Geometry check sheet. Reference: the model listing, model coordinates, mm. Coordinates: 2 decimals unless noted, no trailing zeros. Loops run counter-clockwise (first coordinate to the right, second up) from the corner with the lowest first, then second, coordinate; pieces in that order, holes last. Notation, with made-up numbers: M 18.25,53.25 L 45.25,53.25 A19 ccw 45.25,70.25 Z; hole C 48,20.25 d4. An arc over 180 degrees is marked long. Use CSV: the item, a comma, the result in double quotes.
```python
from build123d import *

# Parameters (mm, degrees)
SKETCH1_W              = 900
SKETCH1_H              = 110
BOSS_EXTRUDE1_DEPTH    = 30
CHAMFER1_SIZE          = 10
CHAMFER2_SIZE          = 15
CHAMFER2_SIZE2         = 10
M16_TAPPED_HOLE1_D     = 14
M16_TAPPED_HOLE1_DEPTH = 45
M16_TAPPED_HOLE1_TIP   = 4.206024333


with BuildPart() as part:
    # Sketch1 → Boss-Extrude1 (new body)
    with BuildSketch(Plane.XY):
        with Locations((450, 55)):
            Rectangle(SKETCH1_W, SKETCH1_H)
    extrude(amount=BOSS_EXTRUDE1_DEPTH)

    # Chamfer1
    chamfer1_edges = [part.edges().sort_by_distance(p)[0] for p in [
        (450, 110, 30),
        (450, 0, 30),
    ]]
    chamfer(chamfer1_edges, length=CHAMFER1_SIZE)

    # Chamfer2
    chamfer2_edges = [part.edges().sort_by_distance(p)[0] for p in [
        (0, 55, 30),
    ]]
    chamfer2_side = [part.faces().sort_by_distance(p)[0] for p in [
        (0, 55, 14.635416667),
    ]]
    chamfer(chamfer2_edges, length=CHAMFER2_SIZE, length2=CHAMFER2_SIZE2, reference=chamfer2_side[0])

    # M16 Tapped Hole1
    with Locations(Plane(origin=(900, 55, 15), x_dir=(0, 0, 1), z_dir=(1, 0, 0))):
        with Locations((0, 0)):
            Hole(M16_TAPPED_HOLE1_D / 2, depth=M16_TAPPED_HOLE1_DEPTH)
            with Locations((0, 0, -(M16_TAPPED_HOLE1_DEPTH + M16_TAPPED_HOLE1_TIP / 2))):  # 118° drill point
                Cone(0, M16_TAPPED_HOLE1_D / 2, M16_TAPPED_HOLE1_TIP, mode=Mode.SUBTRACT)


solid = part.part
```
1. Section check A-A, the plane x = 424.5. Record the cut outline in (y, z), plus the area to 3 significant figures.
The answers:
outline,"M 0,0 L 110,0 L 110,20 L 100,30 L 10,30 L 0,20 Z"
area,"3,200 mm^2"
2. Release check for a two-part mould opening along Z. For faces 1 (the cylindrical face through (877.18, 48.06, 15.91)), 2 (the flat face through (449, 56, 30)), 3 (the flat face through (444, 0, 10)) record: +Z half, -Z half, draft (parallel to the pull), parting line (faces both ways), or undercut.
The answers:
face 1,"undercut"
face 2,"+Z half"
face 3,"draft"
3. Thickness scan on line 1 (Z direction, x = 890.5, y = 55); line 2 (Y direction, x = 873, z = 15); line 3 (Y direction, x = 797, z = 23). Record the ranges inside material, lowest first. Write a range as [from, to].
The answers:
line 1,"[0, 8], [22, 30]"
line 2,"[0, 48], [62, 110]"
line 3,"[3, 107]"
4. Gauge pin test, flat ends, axial feed: P1, Ø6, axis at y = 70, z = 25, coming from the -X side; P2, Ø5, axis at x = 517, z = 23, coming from the -Y side. Record the tip position at first contact, or that the pin passes through.
The answers:
P1,"x = 4.67"
P2,"y = 0.5"
